Check sheet for the modelled part. Datum: model origin and axes. Units: mm. Face numbers are marked on the shaded views. A direction names the side the tool comes from. Round coordinates to 2 decimals unless told otherwise and drop trailing zeros. Order: outer loops, then holes, each group sorted by start corner. A loop starts at its lowest first (then second) coordinate and runs counter-clockwise, first axis right, second up. Notation, with made-up numbers: (41.25, 58.25) -> (74.25, 58.25) arc R22 cw to (74.25, 65.25) -> close; hole circle Ø4 at (18, -22.5). An arc over 180 degrees is marked (long way). Answer in a Markdown table with one row per item. Add a question column.
1. Sectioned sample at D-D, the plane x = 333. Record the boundary of the cut face in (y, z).
2. Sectioned sample at B-B, the plane y = 16. Record the boundary of the cut face in (x, z).
3. Depth check by flat-ended pin: P1, Ø4, axis at y = -3.5, z = 12.5, coming from the -X side; P2, Ø2, axis at x = 287.5, y = 4, coming from the -Z side; P3, Ø2, axis at y = -1.5, z = -13, coming from the +X side. Enter the tip coordinate at first touch or a pass-through.
4. Material ranges on L1, parallel to X at y = 15.5, z = -11; L2, parallel to Z at x = 88, y = -6; L3, parallel to Y at x = 12.5, z = -2.5, recorded low to high. Write a range as from..to.
5. Sectioned sample at A-A, the plane x = 214. Record the boundary of the cut face in (y, z).
6. Access from +Z, -Z, +X, -X, +Y, -Y to the whole of each face (thin tool, end or side, straight path). Record for the marked faces 1, 2 and 3.
7. Sectioned sample at C-C, the plane z = -20.5. Record the boundary of the cut face in (x, y), then the cut area to 3 significant figures.
```python
from build123d import *

# Parameters (mm, degrees)
CUT_EXTRUDE1_DEPTH      = 17
CUT_EXTRUDE1_DEPTH_BACK = 17
CUT_EXTRUDE2_DEPTH      = 17
CUT_EXTRUDE2_DEPTH_BACK = 17
CUT_EXTRUDE3_DEPTH      = 17
CUT_EXTRUDE3_DEPTH_BACK = 17
CUT_EXTRUDE4_DEPTH      = 17
CUT_EXTRUDE4_DEPTH_BACK = 17


with BuildPart() as part:
    # Sketch1 → Revolve1 (revolve)
    with BuildSketch(Plane.XY, mode=Mode.PRIVATE) as revolve1_sk:
        Polygon((-57, 0), (-57, 7.08), (-56.08, 8), (-25, 8), (-23, 10), (133, 10), (133, 24.75), (160, 24.75), (160, 0), align=None)
    revolve(revolve1_sk.sketch.rotate(Axis((160, 0, 0), (-1, 0, 0)), 270), axis=Axis((160, 0, 0), (-1, 0, 0)))

    # Sketch2 → Cut-Extrude1 (cut, two sides: drawn at the far end of the back side and taken through both)
    with BuildSketch(Plane(origin=(0, 0, 0), x_dir=(1, 0, 0), z_dir=(0, -0.7071067811865475, 0.7071067811865476)).offset(-CUT_EXTRUDE1_DEPTH_BACK)):
        Polygon((-74, -25.5), (-1, -25.5), (-18, -8.5), (-57, -8.5), (-57, 8.5), (-18, 8.5), (-1, 25.5), (-74, 25.5), align=None)
    extrude(amount=CUT_EXTRUDE1_DEPTH + CUT_EXTRUDE1_DEPTH_BACK, mode=Mode.SUBTRACT)

    # Sketch3 → Cut-Extrude2 (cut, two sides: drawn at the far end of the back side and taken through both)
    with BuildSketch(Plane(origin=(0, 0, 0), x_dir=(-1, 0, 0), z_dir=(0, -0.7071067811865476, -0.7071067811865475)).offset(-CUT_EXTRUDE2_DEPTH_BACK)):
        Polygon((74, 25.5), (1, 25.5), (18, 8.5), (57, 8.5), (57, -8.5), (18, -8.5), (1, -25.5), (74, -25.5), align=None)
    extrude(amount=CUT_EXTRUDE2_DEPTH + CUT_EXTRUDE2_DEPTH_BACK, mode=Mode.SUBTRACT)

    # Sketch4 → Revolve2 (revolve)
    with BuildSketch(Plane.XY, mode=Mode.PRIVATE) as revolve2_sk:
        Polygon((119, 0), (119, 10), (314, 10), (316, 8), (385.773, 8), (387, 6.773), (387, 0), align=None)
    revolve(revolve2_sk.sketch.rotate(Axis((387, 0, 0), (-1, 0, 0)), 270), axis=Axis((387, 0, 0), (-1, 0, 0)))

    # Sketch5 → Cut-Extrude3 (cut, two sides: drawn at the far end of the back side and taken through both)
    with BuildSketch(Plane(origin=(0, 0, 0), x_dir=(1, 0, 0), z_dir=(0, -0.7071067811865475, 0.7071067811865476)).offset(-CUT_EXTRUDE3_DEPTH_BACK)):
        Polygon((307.5, -10), (307.5, -17), (392, -17), (392, 17), (307.5, 17), (307.5, 10), (309, 8.5), (388, 8.5), (388, -8.5), (309, -8.5), align=None)
    extrude(amount=CUT_EXTRUDE3_DEPTH + CUT_EXTRUDE3_DEPTH_BACK, mode=Mode.SUBTRACT)

    # Sketch6 → Cut-Extrude4 (cut, two sides: drawn at the far end of the back side and taken through both)
    with BuildSketch(Plane(origin=(0, 0, 0), x_dir=(-1, 0, 0), z_dir=(0, -0.7071067811865476, -0.7071067811865475)).offset(-CUT_EXTRUDE4_DEPTH_BACK)):
        Polygon((-307.5, 10), (-307.5, 17), (-392, 17), (-392, -17), (-307.5, -17), (-307.5, -10), (-309, -8.5), (-388, -8.5), (-388, 8.5), (-309, 8.5), align=None)
    extrude(amount=CUT_EXTRUDE4_DEPTH + CUT_EXTRUDE4_DEPTH_BACK, mode=Mode.SUBTRACT)


solid = part.part
```
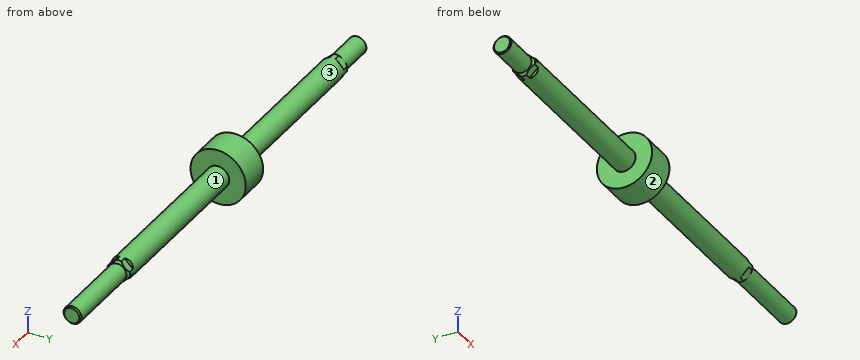
Answer key:
| question | item | result |
|---|---|---|
| 1 | outline | circle Ø16 at (0, 0) |
| 2 | outline | (133, -18.88) -> (160, -18.88) -> (160, 18.88) -> (133, 18.88) -> close |
| 3 | P1 | stops at x = 133 |
| 3 | P2 | stops at z = -9.54 |
| 3 | P3 | stops at x = 160 |
| 4 | L1 | x = 133..160 |
| 4 | L2 | z = -8..8 |
| 4 | L3 | y = -9.68..9.68 |
| 5 | outline | circle Ø20 at (0, 0) |
| 6 | face 1 | +X |
| 6 | face 2 | +X, -X |
| 6 | face 3 | -X |
| 7 | outline | (133, -13.87) -> (160, -13.87) -> (160, 13.87) -> (133, 13.87) -> close |
| 7 | area | 749 mm² |
